from build123d import *

# Parameters (mm, degrees)
FLANGE_PROFILE_SKETCH_R       = 4
SQUARE_FLANGE_100X16_DEPTH    = 16
RECESS_SKETCH_64_R            = 32
RECESS_64X10_DEPTH            = 10
HUB_BOSS_28_REACH             = 70.615
HUB_SKETCH_28_R               = 14
HUB_BOSS_28_DIRECTION_2_DEPTH = 40
HUB_FILLET_R3_R               = 3
KEYED_BORE_DEPTH              = 85.308955633
ARC_SLOTS_REACH               = 80.791


with BuildPart() as part:
    # Flange Profile Sketch → Square Flange 100x16 (new body)
    with BuildSketch(Plane(origin=(0, 0, 0), x_dir=(1, 0, 0), z_dir=(0, 1, 0))):
        with BuildLine():
            ThreePointArc((43.977933562, -6.940896525), (48, 0), (43.977933562, 6.940896525))
            ThreePointArc((43.977933562, 6.940896525), (22.991424972, 22.991424972), (6.940896525, 43.977933562))
            ThreePointArc((6.940896525, 43.977933562), (0, 48), (-6.940896525, 43.977933562))
            ThreePointArc((-6.940896525, 43.977933562), (-22.991424972, 22.991424972), (-43.977933562, 6.940896525))
            ThreePointArc((-43.977933562, 6.940896525), (-48, 0), (-43.977933562, -6.940896525))
            ThreePointArc((-43.977933562, -6.940896525), (-22.991424972, -22.991424972), (-6.940896525, -43.977933562))
            ThreePointArc((-6.940896525, -43.977933562), (0, -48), (6.940896525, -43.977933562))
            ThreePointArc((6.940896525, -43.977933562), (22.991424972, -22.991424972), (43.977933562, -6.940896525))
        make_face()
        with Locations(Location((40, 0, 0), (0, 0, 270))):
            Circle(FLANGE_PROFILE_SKETCH_R, mode=Mode.SUBTRACT)
        with Locations(Location((0, -40, 0), (0, 0, 270))):
            Circle(FLANGE_PROFILE_SKETCH_R, mode=Mode.SUBTRACT)
        with Locations(Location((-40, 0, 0), (0, 0, 270))):
            Circle(FLANGE_PROFILE_SKETCH_R, mode=Mode.SUBTRACT)
        with Locations(Location((0, 40, 0), (0, 0, 270))):
            Circle(FLANGE_PROFILE_SKETCH_R, mode=Mode.SUBTRACT)
    extrude(amount=SQUARE_FLANGE_100X16_DEPTH)

    # Recess Sketch Ø64 → Recess Ø64x10 (cut)
    with BuildSketch(Plane(origin=(0, 16, 0), x_dir=(1, 0, 0), z_dir=(0, 1, 0))):
        with Locations(Location((0, 0, 0), (0, 0, 270))):
            Circle(RECESS_SKETCH_64_R)
    extrude(amount=-RECESS_64X10_DEPTH, mode=Mode.SUBTRACT)

    # Hub Boss Ø28: up to this face of the body (flat: up to its plane)
    hub_boss_28_end = Plane(part.part.faces().sort_by_distance((22.895424972, 16, 22.895424972))[0])
    # Hub Sketch Ø28 → Hub Boss Ø28 (add, up to the picked face)
    with BuildSketch(Plane(origin=(0, 6, 0), x_dir=(1, 0, 0), z_dir=(0, 1, 0)), mode=Mode.PRIVATE) as hub_boss_28_sk1:
        with Locations(Location((0, 0, 0), (0, 0, 270))):
            Circle(HUB_SKETCH_28_R)
    hub_boss_28_tool1 = split(extrude(hub_boss_28_sk1.sketch, amount=HUB_BOSS_28_REACH, mode=Mode.PRIVATE), bisect_by=hub_boss_28_end, keep=Keep.BOTH, mode=Mode.PRIVATE)
    add(hub_boss_28_tool1.solids().sort_by(Axis((0, 6, 0), (0, 1, 0)))[0])

    # Hub Sketch Ø28 → Hub Boss Ø28 direction 2 (add)
    with BuildSketch(Plane(origin=(0, 6, 0), x_dir=(1, 0, 0), z_dir=(0, 1, 0))):
        with Locations(Location((0, 0, 0), (0, 0, 270))):
            Circle(HUB_SKETCH_28_R)
    extrude(amount=-HUB_BOSS_28_DIRECTION_2_DEPTH)

    # Hub Fillet R3
    hub_fillet_r3_edges = [part.edges().sort_by_distance(p)[0] for p in [
        (0, 0, -14),
    ]]
    fillet(hub_fillet_r3_edges, radius=HUB_FILLET_R3_R)

    # Keyed Bore Sketch → Keyed Bore (cut, through all)
    with BuildSketch(Plane(origin=(0, 16, 0), x_dir=(1, 0, 0), z_dir=(0, 1, 0))):
        with BuildLine():
            Line((9.611830035, 0), (9.611830035, 1.937522775))
            Line((9.611830035, 1.937522775), (7.761830035, 1.937522775))
            ThreePointArc((7.761830035, 1.937522775), (-7.999816529, 0.054180315), (7.73487471, -2.042477225))
            Line((7.73487471, -2.042477225), (9.611830035, -2.042477225))
            Line((9.611830035, -2.042477225), (9.611830035, 0))
        make_face()
    extrude(amount=-KEYED_BORE_DEPTH, mode=Mode.SUBTRACT)

    # Arc Slots Sketch → Arc Slots (cut, up to next)
    with BuildSketch(Plane(origin=(0, 6, 0), x_dir=(1, 0, 0), z_dir=(0, 1, 0)), mode=Mode.PRIVATE) as arc_slots_sk1:
        with BuildLine():
            ThreePointArc((18.384776311, 18.384776311), (0, 26), (-18.384776311, 18.384776311))
            ThreePointArc((-18.384776311, 18.384776311), (-18.384776311, 14.142135624), (-14.142135624, 14.142135624))
            ThreePointArc((-14.142135624, 14.142135624), (0, 20), (14.142135624, 14.142135624))
            ThreePointArc((14.142135624, 14.142135624), (18.384776311, 14.142135624), (18.384776311, 18.384776311))
        make_face()
    arc_slots_tool1 = extrude(arc_slots_sk1.sketch, amount=-ARC_SLOTS_REACH, mode=Mode.PRIVATE) & part.part
    # Arc Slots Sketch → Arc Slots (cut, up to next)
    with BuildSketch(Plane(origin=(0, 6, 0), x_dir=(1, 0, 0), z_dir=(0, 1, 0)), mode=Mode.PRIVATE) as arc_slots_sk2:
        with BuildLine():
            ThreePointArc((18.384776311, -18.384776311), (0, -26), (-18.384776311, -18.384776311))
            ThreePointArc((-18.384776311, -18.384776311), (-18.384776311, -14.142135624), (-14.142135624, -14.142135624))
            ThreePointArc((-14.142135624, -14.142135624), (0, -20), (14.142135624, -14.142135624))
            ThreePointArc((14.142135624, -14.142135624), (18.384776311, -14.142135624), (18.384776311, -18.384776311))
        make_face()
    arc_slots_tool2 = extrude(arc_slots_sk2.sketch, amount=-ARC_SLOTS_REACH, mode=Mode.PRIVATE) & part.part
    add(arc_slots_tool1.solids().sort_by_distance((0, 6, -20.194527))[0], mode=Mode.SUBTRACT)
    add(arc_slots_tool2.solids().sort_by_distance((0, 6, 20.194527))[0], mode=Mode.SUBTRACT)


solid = part.part
CAD build for the part. Positions are in the model's coordinates, mm. A direction names the side the tool comes from. Round coordinates to 2 decimals unless told otherwise and drop trailing zeros. Write each loop counter-clockwise with the first axis right and the second up, starting at its lowest first coordinate (ties: lowest second). Pieces come first, ordered by that corner, then holes. Notation, with made-up numbers: M 61.5,38.5 L 74.5,38.5 A26 ccw 74.5,71.5 Z; hole C -20,80 d5. An arc over 180 degrees is marked long. Use a Markdown table: item, result. Add a question column.
1. Slice it at B-B on x = 40. Give the cut face in (y, z).
2. Pull direction X, two halves, no side cores. Call faces 1 (the face through (14, 0, 10)), 2 (the face through (0, 3, 20)), 3 (the face through (22.73, 7.888, 23.254)): released by +X, released by -X, zero draft, split by the parting line, or undercut.
3. Slice it at A-A on z = 0. Give the number of separate pieces and of enclosed holes in the cut face, then the cut area to 3 significant figures.
4. Drill centre lines: probe 1 along X at (y, z) = (9.5, 0); probe 2 along X at (y, z) = (4, 0); probe 3 along X at (y, z) = (12.5, 11) (3 decimals). Where is each one in solid material? Low to high.
5. Flat gauge pins, fed straight in: P1, Ø9, axis at x = 40, z = 0, coming from the -Y side; P2, Ø1.5, axis at x = 8.5, y = 3.5, coming from the -Z side; P3, Ø4.5, axis at y = -3.5, z = 0.5, coming from the -X side. Where does each tip first touch, or does it go through?
6. Slice it at C-C on y = -13.5. Give the cut face in (x, z), then the cut area to 3 significant figures.
7. 3-axis set-ups, long thin cutter, end or side, ignore diameter. For faces 4 (the face through (-14, 6, 7)), 5 (the face through (-22.73, 7.888, -23.254)), 6 (the face through (0, 8, -48)), 7 (the face through (0, 3, -26)), 8 (the face through (-13.67, -18.28, -3.03)): which of +Z, -Z, +X, -X, +Y, -Y reach the whole face in a straight line?
Reply:
| question | item | result |
|---|---|---|
| 1 | outline | M 0,-9.35 L 16,-9.35 L 16,-4 L 0,-4 Z; M 0,4 L 16,4 L 16,9.35 L 0,9.35 Z |
| 2 | face 1 | zero draft |
| 2 | face 2 | undercut |
| 2 | face 3 | released by +X |
| 3 | separate pieces | 4 |
| 3 | enclosed holes | 0 |
| 3 | area | 995 mm^2 |
| 4 | probe 1 | x = -48 to -44, -36 to -32, -14 to -8, 9.61 to 14, 32 to 36, 44 to 48 |
| 4 | probe 2 | x = -48 to -44, -36 to -8, 9.61 to 36, 44 to 48 |
| 4 | probe 3 | x = -37.485 to -30.05, -8.66 to 8.66, 30.05 to 37.485 |
| 5 | P1 | stops at y = 0 |
| 5 | P2 | stops at z = -42.59 |
| 5 | P3 | stops at x = -14.56 |
| 6 | outline | C 0,0 d28; hole M 7.73,2.04 A8 ccw long 7.76,-1.94 L 9.61,-1.94 L 9.61,2.04 Z |
| 6 | area | 408 mm^2 |
| 7 | face 4 | +Y |
| 7 | face 5 | -Z, -X, +Y, -Y |
| 7 | face 6 | -Z, +Y, -Y |
| 7 | face 7 | +Y, -Y |
| 7 | face 8 | -Y |
